The model under review builds one solid part; all positions refer to its coordinate system, in mm. Face numbers are marked on the shaded views. A direction names the side the tool comes from. Round coordinates to 2 decimals unless told otherwise and drop trailing zeros. Loops run counter-clockwise (first coordinate to the right, second up) from the corner with the lowest first, then second, coordinate; pieces in that order, holes last. Notation, with made-up numbers: (19, -14) -> (34, -14) arc R23 cw to (34, 9) -> close; hole circle Ø10 at (38, 50). An arc over 180 degrees is marked (long way). Use a Markdown table: item, result. Add a question column.
1) Insertion check: pin 1 (6 mm diameter, centred on y = 37.5, z = -7.5, fed in from +X); pin 2 (2 mm diameter, centred on y = 37.5, z = -25.5, fed in from -X); pin 3 (1.5 mm diameter, centred on x = 3.5, z = -12, fed in from -Y). Each pin has a flat end and moves straight along its axis. Give the tip position at first contact, or say it passes through.
2) Consider section C-C on x = 8. Give the boundary of the cut face in (y, z).
3) Wall thickness on probe 1 along Z at (x, y) = (5, 6); probe 2 along Y at (x, z) = (7.8, -21); probe 3 along X at (y, z) = (43, 13.5): over which ranges is each line inside the solid? List them lowest first.
4) Consider section A-A on y = 36.5. Give the boundary of the cut face in (x, z), plus the area to 3 significant figures.
5) For the marked faces 1, 2 and 3, list the 3-axis set-ups (+Z, -Z, +X, -X, +Y, -Y) from which the entire face can be reached by the end or side of a thin tool; tool diameter is ignored.
6) Consider section D-D on y = 4. Give the boundary of the cut face in (x, z).
7) Consider section B-B on z = -21.5. Give the boundary of the cut face in (x, y).
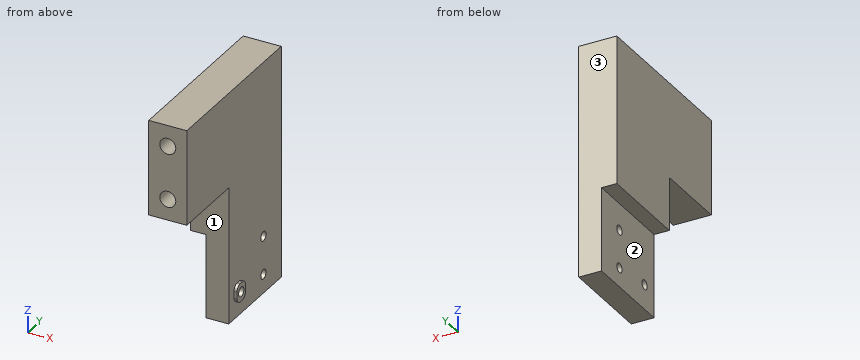
from build123d import *

# Parameters (mm, degrees)
EXTRUDE_THIN1_DEPTH   = 25
SKETCH2_W             = 36
SKETCH2_H             = 25
BOSS_EXTRUDE1_DEPTH   = 10
SKETCH5_W             = 4
SKETCH5_H             = 22
CUT_EXTRUDE1_DEPTH    = 68.424031324
SKETCH6_W             = 93.972678959
SKETCH6_H             = 54.427614962
CUT_EXTRUDE2_DEPTH    = 10
M5_TAPPED_HOLE1_D     = 4.2
M5_TAPPED_HOLE1_DEPTH = 12.4
M5_TAPPED_HOLE1_TIP   = 1.2618073
M3_TAPPED_HOLE1_D     = 2.5
SKETCH12_W            = 4.8
SKETCH12_H            = 4
BOSS_EXTRUDE2_DEPTH   = 0.8
M3_TAPPED_HOLE2_D     = 2.5
FILLET1_R             = 1.5


with BuildPart() as part:
    # Sketch1 → Extrude-Thin1 (new body)
    with BuildSketch(Plane.XY):
        Polygon((-15, 0), (0, 0), (0, 45), (10, 45), (10, -10), (-15, -10), align=None)
    extrude(amount=EXTRUDE_THIN1_DEPTH)

    # Sketch2 → Boss-Extrude1 (add)
    with BuildSketch(Plane.ZY):
        with Locations((-18, 32.5)):
            Rectangle(SKETCH2_W, SKETCH2_H)
    extrude(amount=-BOSS_EXTRUDE1_DEPTH)

    # Sketch5 → Cut-Extrude1 (cut, through all)
    with BuildSketch(Plane(origin=(0, 45, 0), x_dir=(1, 0, 0), z_dir=(0, 1, 0))):
        with Locations((2, 25)):
            Rectangle(SKETCH5_W, SKETCH5_H)
    extrude(amount=-CUT_EXTRUDE1_DEPTH, mode=Mode.SUBTRACT)

    # Sketch6 → Cut-Extrude2 (cut)
    with BuildSketch(Plane.XZ.offset(10)):
        with Locations((-13.059524258, 16.160355611)):
            Rectangle(SKETCH6_W, SKETCH6_H)
    extrude(amount=-CUT_EXTRUDE2_DEPTH, mode=Mode.SUBTRACT)

    # M5 Tapped Hole1
    with Locations(Plane(origin=(0, 0, 0), x_dir=(-1, 0, 0), z_dir=(0, -1, 0))):
        with Locations((-5, -5.5), (-5, -19.5)):
            Hole(M5_TAPPED_HOLE1_D / 2, depth=M5_TAPPED_HOLE1_DEPTH)
            with Locations((0, 0, -(M5_TAPPED_HOLE1_DEPTH + M5_TAPPED_HOLE1_TIP / 2))):  # 118° drill point
                Cone(0, M5_TAPPED_HOLE1_D / 2, M5_TAPPED_HOLE1_TIP, mode=Mode.SUBTRACT)

    # M3 Tapped Hole1 (through all)
    with Locations(Plane(origin=(10, 0, 0), x_dir=(0, 0, -1), z_dir=(1, 0, 0))):
        with Locations((21, 36.5), (31, 36.5)):
            Hole(M3_TAPPED_HOLE1_D / 2)

    # Sketch12 → Boss-Extrude2 (add)
    with BuildSketch(Plane(origin=(10, 0, 0), x_dir=(0, 0, -1), z_dir=(1, 0, 0))):
        with Locations((29.5, 24.5)):
            Rectangle(SKETCH12_W, SKETCH12_H)
    extrude(amount=BOSS_EXTRUDE2_DEPTH)

    # M3 Tapped Hole2 (through all)
    with Locations(Plane.ZY):
        with Locations((-29.5, 24.5)):
            Hole(M3_TAPPED_HOLE2_D / 2)

    # Fillet1
    fillet1_edges = [part.edges().sort_by_distance(p)[0] for p in [
        (10.4, 22.5, -31.9),
        (10.4, 26.5, -31.9),
        (10.4, 26.5, -27.1),
        (10.4, 22.5, -27.1),
    ]]
    fillet(fillet1_edges, radius=FILLET1_R)


solid = part.part
Result set:
| question | item | result |
|---|---|---|
| 1 | pin 1 | x = 10 |
| 1 | pin 2 | x = 4 |
| 1 | pin 3 | y = 20 |
| 2 | outline | (0, 0) -> (20, 0) -> (20, -36) -> (45, -36) -> (45, 25) -> (0, 25) -> close; hole circle Ø2.5 at (24.5, -29.5); hole circle Ø2.5 at (36.5, -31); hole circle Ø2.5 at (36.5, -21) |
| 3 | probe 1 | 0 to 3.4, 7.6 to 17.4, 21.6 to 25 |
| 3 | probe 2 | 20 to 35.25, 37.75 to 45 |
| 3 | probe 3 | 0 to 10 |
| 4 | outline | (0, -14) -> (4, -14) -> (4, -19.75) -> (10, -19.75) -> (10, 25) -> (0, 25) -> close; (4, -36) -> (10, -36) -> (10, -32.25) -> (4, -32.25) -> close; (4, -29.75) -> (10, -29.75) -> (10, -22.25) -> (4, -22.25) -> close |
| 4 | area | 492 mm2 |
| 5 | face 1 | -Z, +X, -X, -Y |
| 5 | face 2 | -Z, -X, +Y, -Y |
| 5 | face 3 | +Z, -Z, +X, -X, +Y |
| 6 | outline | (0, 0) -> (10, 0) -> (10, 25) -> (0, 25) -> close; hole circle Ø4.2 at (5, 5.5); hole circle Ø4.2 at (5, 19.5) |
| 7 | outline | (4, 20) -> (10, 20) -> (10, 35.35) -> (4, 35.35) -> close; (4, 37.65) -> (10, 37.65) -> (10, 45) -> (4, 45) -> close |
